```python
from build123d import *

# Parameters (mm, degrees)
SWEEP_THIN1_PROFILE_R   = 15
SWEEP_THIN1_PROFILE_R_2 = 13


with BuildPart() as part:
    # Sweep-Thin1: sweep along a path in Sketch1
    with BuildLine(Plane.XY) as sweep_thin1_path:
        Line((200, 0), (40, 0))
        ThreePointArc((40, 0), (11.715728753, 11.715728753), (0, 40))
        Line((0, 40), (0, 502))
    # Sweep-Thin1 profile (on start of the path) → Sweep-Thin1 (sweep)
    with BuildSketch(Plane(origin=(200, 0, 0), x_dir=(0, 0, -1), z_dir=(-1, 0, 0))):
        Circle(SWEEP_THIN1_PROFILE_R)
        Circle(SWEEP_THIN1_PROFILE_R_2, mode=Mode.SUBTRACT)
    sweep(path=sweep_thin1_path.line)


solid = part.part
```
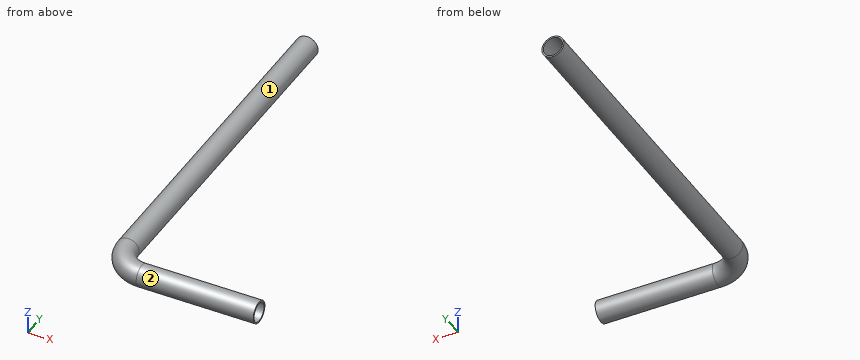
Here's how the part is built. I have some questions about the finished solid (model axes, mm). Face numbers are marked on the shaded views. A direction names the side the tool comes from. Give positions to 0.01 mm unless a question says otherwise; leave off trailing zeros. Loops run counter-clockwise (first coordinate to the right, second up) from the corner with the lowest first, then second, coordinate; pieces in that order, holes last. Notation, with made-up numbers: (32, 9) -> (66, 9) arc R7 cw to (66, 22) -> close; hole circle Ø1 at (-8.5, 76). An arc over 180 degrees is marked (long way). Use one line per item in the form item = value. Start each with the question number.
1) For P1, Ø1, axis at x = 140, z = -11.5, coming from the +Y side; P2, Ø5, axis at x = 56.5, z = -3.5, coming from the +Y side; P3, Ø1.5, axis at x = 159.5, z = -11, coming from the -Y side, each with a flat end and sliding along its axis, tell me the tip position at first contact or that it passes through.
2) Imagine slicing it at A-A (z = 0). Please give me the cut outline in (x, y).
3) Imagine slicing it at B-B (y = 154). Please give me the cut outline in (x, z), then the cut area to 3 significant figures.
4) Which directions (+Z, -Z, +X, -X, +Y, -Y) give clear straight access to the entire face, cutting with the end or side of a thin tool? Please do the marked faces 1 and 2.
5) Please list where these lines run through material, in increasing order: line 1 along X through (y, z) = (313.5, 0); line 2 along X through (y, z) = (280, 6).
Check values:
q1.P1 = 10.2
q1.P2 = 14.97
q1.P3 = -10.95
q2.outline = (-15, 40) arc R55 ccw to (40, -15) -> (200, -15) -> (200, -13) -> (40, -13) arc R53 cw to (-13, 40) -> (-13, 502) -> (-15, 502) -> close; (13, 40) arc R27 ccw to (40, 13) -> (200, 13) -> (200, 15) -> (40, 15) arc R25 cw to (15, 40) -> (15, 502) -> (13, 502) -> close
q3.outline = circle Ø30 at (0, 0); hole circle Ø26 at (0, 0)
q3.area = 176 mm^2
q4.face_1 = +Y
q4.face_2 = +X
q5.line_1 = -15 to -13, 13 to 15
q5.line_2 = -13.75 to -11.53, 11.53 to 13.75
